from build123d import *

# Parameters (mm, degrees)
BOSS_EXTRUDE1_DEPTH                                  = 8
CUT_EXTRUDE2_DEPTH                                   = 24.366642891
M4_TAPPED_HOLE1_D                                    = 3.3
M4_TAPPED_HOLE1_DEPTH                                = 11.5
M4_TAPPED_HOLE1_TIP                                  = 0.991420021
HOLE_SIZE_PER_SOCKET_HEAD_CAP_SCREW_TYPE_D           = 4.5
HOLE_SIZE_PER_SOCKET_HEAD_CAP_SCREW_TYPE_CBORE_D     = 8
HOLE_SIZE_PER_SOCKET_HEAD_CAP_SCREW_TYPE_CBORE_DEPTH = 5
CHAMFER2_SIZE                                        = 1


with BuildPart() as part:
    # Sketch1 → Boss-Extrude1 (new, symmetric)
    with BuildSketch(Plane(origin=(0, 0, 0), x_dir=(1, 0, 0), z_dir=(0, 1, 0))):
        with BuildLine():
            Line((-7.922147119, -39), (7.922147119, -39))
            Line((7.922147119, -39), (19, -34.967991292))
            Line((19, -34.967991292), (19, -28))
            Line((19, -28), (15.491933385, -28))
            ThreePointArc((15.491933385, -28), (0, -32), (-15.491933385, -28))
            Line((-15.491933385, -28), (-19, -28))
            Line((-19, -28), (-19, -34.967991292))
            Line((-19, -34.967991292), (-7.922147119, -39))
        make_face()
    extrude(amount=BOSS_EXTRUDE1_DEPTH, both=True)

    # Sketch2 → Cut-Extrude2 (cut, through all)
    with BuildSketch(Plane.XY.offset(39)):
        Polygon((4.099186911, -2), (2.049593456, 1.55), (-2.049593456, 1.55), (-4.099186911, -2), (-2.049593456, -5.55), (2.049593456, -5.55), align=None)
    extrude(amount=-CUT_EXTRUDE2_DEPTH, mode=Mode.SUBTRACT)

    # M4 Tapped Hole1
    with Locations(Plane(origin=(0, 8, 0), x_dir=(1, 0, 0), z_dir=(0, 1, 0))):
        with Locations((0, -35.5)):
            Hole(M4_TAPPED_HOLE1_D / 2, depth=M4_TAPPED_HOLE1_DEPTH)
            with Locations((0, 0, -(M4_TAPPED_HOLE1_DEPTH + M4_TAPPED_HOLE1_TIP / 2))):  # 118° drill point
                Cone(0, M4_TAPPED_HOLE1_D / 2, M4_TAPPED_HOLE1_TIP, mode=Mode.SUBTRACT)

    # Hole size per socket head cap screw type 2 (through all)
    with Locations(Plane(origin=(-13.461073559, 0, 36.983995646), x_dir=(0.9396926207859081, 0, 0.34202014332566943), z_dir=(-0.34202014332566943, 0, 0.9396926207859081))):
        with Locations((0, 0)):
            hole_size_per_socket_head_cap_screw_type = CounterBoreHole(HOLE_SIZE_PER_SOCKET_HEAD_CAP_SCREW_TYPE_D / 2, HOLE_SIZE_PER_SOCKET_HEAD_CAP_SCREW_TYPE_CBORE_D / 2, HOLE_SIZE_PER_SOCKET_HEAD_CAP_SCREW_TYPE_CBORE_DEPTH)

    # Mirror3: Hole size per socket head cap screw type 2 across plane
    add(hole_size_per_socket_head_cap_screw_type.mirror(Plane(origin=(0, 0, 0), x_dir=(0, 0, 1), z_dir=(1, 0, 0))), mode=Mode.SUBTRACT)

    # Chamfer2
    chamfer2_edges = [part.edges().sort_by_distance(p)[0] for p in [
        (-19, 0, 28),
        (19, 0, 28),
    ]]
    chamfer(chamfer2_edges, length=CHAMFER2_SIZE)


solid = part.part
For this review, take the finished solid that the model builds, in its own axes (mm). A direction names the side the tool comes from. Give positions to 0.01 mm unless a question says otherwise; leave off trailing zeros. Order: outer loops, then holes, each group sorted by start corner. A loop starts at its lowest first (then second) coordinate and runs counter-clockwise, first axis right, second up. Notation, with made-up numbers: M 86.5,46.5 L 119.5,46.5 A9 ccw 119.5,60.5 Z; hole C 48.5,-36.75 d7. An arc over 180 degrees is marked long. Answer in a Markdown table with one row per item. Add a question column.
(1) For pin 1 (3 mm diameter, centred on x = -5.5, y = 5.5, fed in from -Z) (3 decimals); pin 2 (2 mm diameter, centred on x = 0, z = 35.5, fed in from +Y); pin 3 (2 mm diameter, centred on y = -1.5, z = 37.5, fed in from -X), all flat-tipped, find the tip position at first contact; note any pin that passes through.
(2) Wall thickness on probe 1 along X at (y, z) = (-0.5, 33); probe 2 along Z at (x, y) = (0, 3.75); probe 3 along Y at (x, z) = (11.5, 32): over which ranges is each line inside the solid? List them lowest first. Write a range as [from, to].
(3) Mouldability with a two-part tool opening along X and no side actions: class faces 1 (the face through (-18.5, 0.1, 28.5)), 2 (the face through (17, 0, 28)), 3 (the face through (-0.89, 4.73, 34.11)) as +X half, -X half, draft (parallel to the pull), parting line (faces both ways), or undercut.
(4) Consider section B-B on y = -0.75. Give the number of separate pieces and of enclosed holes in the cut face, and give its area (3 significant figures).
(5) For faces 4 (the face through (0, 8, 33)), 5 (the face through (1, 1.55, 37)), 6 (the face through (10.133, -1.722, 32.874)), list the 3-axis set-ups (+Z, -Z, +X, -X, +Y, -Y) from which the entire face can be reached by the end or side of a thin tool; tool diameter is ignored.
(6) Consider section A-A on x = 0. State the section outline as (y, z) points.
Evaluation:
| question | item | result |
|---|---|---|
| 1 | pin 1 | stops at z = 31.225 |
| 1 | pin 2 | stops at y = -5.55 |
| 1 | pin 3 | stops at x = -10.4 |
| 2 | probe 1 | x = [-19, -16.23], [-9.68, -3.23], [3.23, 9.68], [16.23, 19] |
| 2 | probe 2 | z = [32, 33.85], [37.15, 39] |
| 2 | probe 3 | y = [-8, -2.25], [2.25, 8] |
| 3 | face 1 | -X half |
| 3 | face 2 | draft |
| 3 | face 3 | undercut |
| 4 | separate pieces | 4 |
| 4 | enclosed holes | 0 |
| 4 | area | 142 mm^2 |
| 5 | face 4 | +Z, -Z, +X, -X, +Y |
| 5 | face 5 | +Z, -Z |
| 5 | face 6 | none |
| 6 | outline | M -8,32 L -5.55,32 L -5.55,39 L -8,39 Z; M 1.55,32 L 8,32 L 8,33.85 L 1.55,33.85 Z; M 1.55,37.15 L 8,37.15 L 8,39 L 1.55,39 Z |
